Model file for the job. Use its own axes, mm. Face numbers are marked on the shaded views. A direction names the side the tool comes from. Round coordinates to 2 decimals unless told otherwise and drop trailing zeros. Loops run counter-clockwise (first coordinate to the right, second up) from the corner with the lowest first, then second, coordinate; pieces in that order, holes last. Notation, with made-up numbers: M -25.5,-19.5 L 14.5,-19.5 A23 ccw 14.5,15.5 Z; hole C 36,66.25 d7. An arc over 180 degrees is marked long. Use a Markdown table: item, result. Add a question column.
Q1. Cut at C-C (z = 5). Give the cut face in (x, y), plus the area to 3 significant figures.
Q2. Cut at B-B (y = 0). Give the cut face in (x, z), plus the area to 3 significant figures.
Q3. Mould opens along X. For the marked faces 1, 2 and 3 say: +X half, -X half, draft (parallel to the pull), parting line (faces both ways), or undercut.
Q4. Cut at A-A (x = -59.5). Give the cut face in (y, z), plus the area to 3 significant figures.
Q5. Probe line 1 (Y direction, x = -103, z = -7.5); line 2 (Z direction, x = -110, y = 89.5); line 3 (Y direction, x = -85, z = 11). List the from-to ranges inside material, lowest first. Write a range as from..to.
Q6. Pin check, flat tips, straight feed: pin 1 (14.5 mm diameter, centred on x = -100, y = 68, fed in from -Z); pin 2 (2 mm diameter, centred on x = -34, z = -15, fed in from +Y); pin 3 (17.5 mm diameter, centred on y = -7, z = -3, fed in from +X); pin 4 (8 mm diameter, centred on x = 0, z = -1, fed in from -Y). Stop position of each tip, or through.
Q7. Cut at D-D (y = 16). Give the cut face in (x, z), plus the area to 3 significant figures.
Q8. Tool access for the marked faces 4, 5, 6, 7 and 8: list every direction of +Z, -Z, +X, -X, +Y, -Y with a clear straight run to the whole face (end or side of a thin tool).
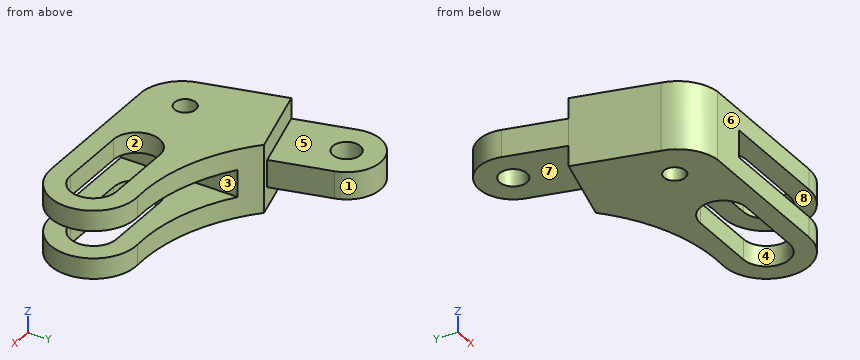
from build123d import *

# Parameters (mm, degrees)
BASE_PLATE_PROFILE_R = 6.25
BASE_PLATE_DEPTH     = 20
GUIDE_SLOT_DEPTH     = 137.100207792
FORK_GAP_16MM_DEPTH  = 8
PIVOT_LUG_DEPTH      = 8
PIVOT_HOLE_PROFILE_R = 8
PIVOT_HOLE_16_DEPTH  = 80


with BuildPart() as part:
    # Base Plate Profile → Base Plate (new, symmetric)
    with BuildSketch(Plane.XY):
        with BuildLine():
            Line((0, -25), (-85, -25))
            ThreePointArc((-85, -25), (-98.929277245, -18.882655563), (-106.733331092, -5.823428515))
            Line((-106.733331092, -5.823428515), (-119.156645256, 40.541011147))
            Line((-119.156645256, 40.541011147), (-75.640400658, 52.201153745))
            ThreePointArc((-75.640400658, 52.201153745), (-41.316083866, 30.926455065), (-1.376154737, 24.962095227))
            ThreePointArc((-1.376154737, 24.962095227), (24.99052201, 0.688338331), (0, -25))
        make_face()
        with Locations((-85, 0)):
            Circle(BASE_PLATE_PROFILE_R, mode=Mode.SUBTRACT)
    extrude(amount=BASE_PLATE_DEPTH, both=True)

    # Guide Slot Profile → Guide Slot (cut, through all)
    with BuildSketch(Plane.XY.offset(20)):
        with BuildLine():
            Line((-40, 13.5), (0, 13.5))
            ThreePointArc((0, 13.5), (13.5, 0), (0, -13.5))
            Line((0, -13.5), (-40, -13.5))
            ThreePointArc((-40, -13.5), (-53.5, 0), (-40, 13.5))
        make_face()
    extrude(amount=-GUIDE_SLOT_DEPTH, mode=Mode.SUBTRACT)

    # Fork Gap Profile → Fork Gap 16mm (cut, symmetric)
    with BuildSketch(Plane.XY):
        with BuildLine():
            Line((-65, 43.433848458), (-65, -25))
            Line((-65, -25), (0, -25))
            ThreePointArc((0, -25), (24.99052201, 0.688338331), (-1.376154737, 24.962095227))
            ThreePointArc((-1.376154737, 24.962095227), (-34.762230676, 28.775980481), (-65, 43.433848458))
        make_face()
    extrude(amount=FORK_GAP_16MM_DEPTH, both=True, mode=Mode.SUBTRACT)

    # Pivot Lug Profile → Pivot Lug (add, symmetric)
    with BuildSketch(Plane.XY):
        with BuildLine():
            Line((-119.156645256, 40.541011147), (-128.215311835, 74.348415067))
            ThreePointArc((-128.215311835, 74.348415067), (-114.073176211, 98.843312495), (-89.578278783, 84.701176871))
            Line((-89.578278783, 84.701176871), (-80.519612205, 50.893772951))
            Line((-80.519612205, 50.893772951), (-119.156645256, 40.541011147))
        make_face()
    extrude(amount=PIVOT_LUG_DEPTH, both=True)

    # Pivot Hole Profile → Pivot Hole Ø16 (cut, symmetric)
    with BuildSketch(Plane.XY.offset(8)):
        with Locations(Location((-108.896795309, 79.524795969, 0), (0, 0, 180))):
            Circle(PIVOT_HOLE_PROFILE_R)
    extrude(amount=PIVOT_HOLE_16_DEPTH, both=True, mode=Mode.SUBTRACT)


solid = part.part
Checked values:
| question | item | result |
|---|---|---|
| 1 | outline | M -128.22,74.35 L -106.73,-5.82 A25 ccw -85,-25 L -65,-25 L -65,43.43 A100 cw -75.64,52.2 L -80.52,50.89 L -89.58,84.7 A20 ccw Z; hole C -108.9,79.52 d16; hole C -85,0 d12.5 |
| 1 | area | 4,940 mm^2 |
| 2 | outline | M -108.29,-20 L -91.25,-20 L -91.25,20 L -108.29,20 Z; M -78.75,-20 L -53.5,-20 L -53.5,-8 L -65,-8 L -65,8 L -53.5,8 L -53.5,20 L -78.75,20 Z; M 13.5,-20 L 25,-20 L 25,-8 L 13.5,-8 Z; M 13.5,8 L 25,8 L 25,20 L 13.5,20 Z |
| 2 | area | 1,780 mm^2 |
| 3 | face 1 | parting line |
| 3 | face 2 | undercut |
| 3 | face 3 | +X half |
| 4 | outline | M -25,-20 L 39.77,-20 L 39.77,-8 L -25,-8 Z; M -25,8 L 39.77,8 L 39.77,20 L -25,20 Z |
| 4 | area | 1,550 mm^2 |
| 5 | line 1 | y = -14.29..74.12, 84.93..98.64 |
| 5 | line 2 | z = -8..8 |
| 5 | line 3 | y = -25..-6.25, 6.25..49.69 |
| 6 | pin 1 | stops at z = -8 |
| 6 | pin 2 | stops at y = 28.85 |
| 6 | pin 3 | stops at x = 25 |
| 6 | pin 4 | passes through |
| 7 | outline | M -112.58,-20 L 19.21,-20 L 19.21,-8 L -65,-8 L -65,8 L 19.21,8 L 19.21,20 L -112.58,20 Z |
| 7 | area | 3,920 mm^2 |
| 8 | face 4 | +Z, -Z |
| 8 | face 5 | +Z, -X, +Y |
| 8 | face 6 | +Z, -Z, +X, -X, -Y |
| 8 | face 7 | -Z, -X, +Y |
| 8 | face 8 | +X, +Y, -Y |
